For this review, take the finished solid that the model builds, in its own axes (mm). Face numbers are marked on the shaded views. A direction names the side the tool comes from. Round coordinates to 2 decimals unless told otherwise and drop trailing zeros. Write each loop counter-clockwise with the first axis right and the second up, starting at its lowest first coordinate (ties: lowest second). Pieces come first, ordered by that corner, then holes. Notation, with made-up numbers: (38.25, -37.5) -> (73.25, -37.5) arc R16 ccw to (73.25, -33.5) -> close; hole circle Ø9 at (46, -10.5). An arc over 180 degrees is marked (long way). Answer in a Markdown table with one row per item.
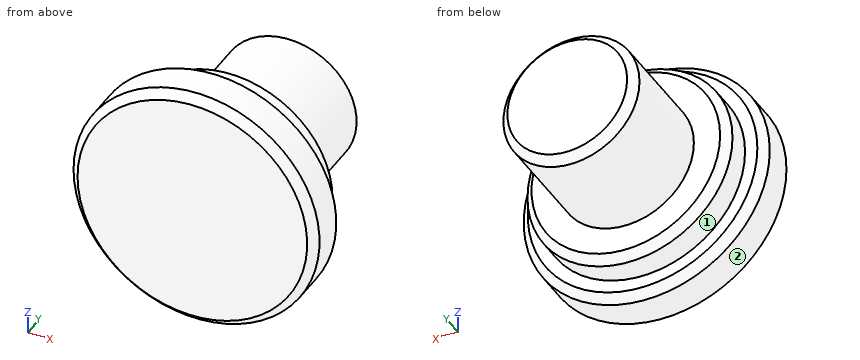
from build123d import *

# Parameters (mm, degrees)
CHAMFER1_SIZE = 0.5


with BuildPart() as part:
    # Sketch1 → Revolve1 (revolve)
    with BuildSketch(Plane.XY, mode=Mode.PRIVATE) as revolve1_sk:
        Polygon((154.87840727, -569.505265962), (152.77840727, -569.505265962), (152.77840727, -562.505265962), (148.62840727, -562.505265962), (148.62840727, -574.505265962), (156.12840727, -574.505265962), (156.12840727, -571.505265962), (154.87840727, -571.505265962), align=None)
    revolve(revolve1_sk.sketch.rotate(Axis((148.62840727, -560.805265962, 0), (0, -1, 0)), 180), axis=Axis((148.62840727, -560.805265962, 0), (0, -1, 0)))

    # Chamfer1
    chamfer1_edges = [part.edges().sort_by_distance(p)[0] for p in [
        (154.87840727, -569.505265962, 0),
        (156.12840727, -571.505265962, 0),
        (156.12840727, -574.505265962, 0),
        (152.77840727, -562.505265962, 0),
    ]]
    chamfer(chamfer1_edges, length=CHAMFER1_SIZE)


solid = part.part
1) Consider section B-B on y = -562.75. State the section outline as (x, z) points, then the cut area to 3 significant figures.
Solved:
| item | result |
|---|---|
| outline | circle Ø7.79 at (148.63, 0) |
| area | 47.7 mm² |
2) For the marked faces 1 and 2, list the 3-axis set-ups (+Z, -Z, +X, -X, +Y, -Y) from which the entire face can be reached by the end or side of a thin tool; tool diameter is ignored.
Solved:
| item | result |
|---|---|
| face 1 | +Y |
| face 2 | +Y, -Y |
3) Clearance check with flat-ended pins moving along their axes: pin 1 Ø3 at (y, z) = (-565, 1) entering from -X; pin 2 Ø4 at (y, z) = (-573, -3.5) entering from -X; pin 3 Ø1.5 at (y, z) = (-570.5, -1.5) entering from +X. State where each tip first meets the part, or that it passes through.
Solved:
| item | result |
|---|---|
| pin 1 | x = 144.48 |
| pin 2 | x = 141.28 |
| pin 3 | x = 154.83 |
4) Consider section C-C on y = -565.75. State the section outline as (x, z) points.
Solved:
| item | result |
|---|---|
| outline | circle Ø8.3 at (148.63, 0) |
5) For line 1 (Y direction, x = 142.25, z = 1); line 2 (Y direction, x = 152, z = 2.5); line 3 (Z direction, x = 151.5, y = -570.25), list the stretches that pass through material, from the lowest coordinate up. Write a range as [from, to].
Solved:
| item | result |
|---|---|
| line 1 | [-574.51, -571.51] |
| line 2 | [-574.51, -569.51] |
| line 3 | [-5.55, 5.55] |
6) Consider section A-A on z = 0. State the section outline as (x, y) points, then the cut area to 3 significant figures.
Solved:
| item | result |
|---|---|
| outline | (141.13, -574.01) -> (141.63, -574.51) -> (155.63, -574.51) -> (156.13, -574.01) -> (156.13, -572.01) -> (155.63, -571.51) -> (154.88, -571.51) -> (154.88, -570.01) -> (154.38, -569.51) -> (152.78, -569.51) -> (152.78, -563.01) -> (152.28, -562.51) -> (144.98, -562.51) -> (144.48, -563.01) -> (144.48, -569.51) -> (142.88, -569.51) -> (142.38, -570.01) -> (142.38, -571.51) -> (141.63, -571.51) -> (141.13, -572.01) -> close |
| area | 127 mm² |
